```python
from build123d import *

# Parameters (mm, degrees)
SKETCH1_R                  = 50
BOSS_EXTRUDE1_DEPTH        = 20
M56X4_0_TAPPED_HOLE1_D     = 52
M56X4_0_TAPPED_HOLE1_DEPTH = 124
M56X4_0_TAPPED_HOLE1_TIP   = 15.622376095
CIRPATTERN1_COUNT          = 4


with BuildPart() as part:
    # Sketch1 → Boss-Extrude1 (new body)
    with BuildSketch(Plane(origin=(0, 0, 0), x_dir=(1, 0, 0), z_dir=(0, 1, 0))):
        with Locations(Location((0, 0, 0), (0, 0, 270))):
            Circle(SKETCH1_R)
    extrude(amount=BOSS_EXTRUDE1_DEPTH)

    # M56x4.0 Tapped Hole1
    with Locations(Plane(origin=(0, 20, 0), x_dir=(1, 0, 0), z_dir=(0, 1, 0))):
        with Locations((0, 0)):
            Hole(M56X4_0_TAPPED_HOLE1_D / 2, depth=M56X4_0_TAPPED_HOLE1_DEPTH)
            with Locations((0, 0, -(M56X4_0_TAPPED_HOLE1_DEPTH + M56X4_0_TAPPED_HOLE1_TIP / 2))):  # 118° drill point
                Cone(0, M56X4_0_TAPPED_HOLE1_D / 2, M56X4_0_TAPPED_HOLE1_TIP, mode=Mode.SUBTRACT)

    # Sketch5 → Ø14.0 (14) Diameter Hole1 (revolve, cut)
    with BuildSketch(Plane(origin=(0, 10, 50), x_dir=(0, -1, 0), z_dir=(1, 0, 0))):
        Polygon((0, 0), (0, 20), (7, 15.793975667), (7, 0), align=None)
    f_14_0_14_diameter_hole1 = revolve(axis=Axis((0, 10, 56.35), (0, 0, -1)), mode=Mode.SUBTRACT)

    # CirPattern1: Ø14.0 (14) Diameter Hole1 ×4 about axis
    cirpattern1_axis = Axis((0, 20, 0), (0, 1, 0))
    for i in range(1, CIRPATTERN1_COUNT):
        add(f_14_0_14_diameter_hole1.rotate(cirpattern1_axis, i * 360 / CIRPATTERN1_COUNT), mode=Mode.SUBTRACT)


solid = part.part
```
Verification items for the finished model (mm, model axes). A direction names the side the tool comes from. Give positions to 0.01 mm unless a question says otherwise; leave off trailing zeros. Loops run counter-clockwise (first coordinate to the right, second up) from the corner with the lowest first, then second, coordinate; pieces in that order, holes last.
1. Section check C-C, the plane z = 13.5. Enter the section's corners in (x, y), then the cut area to 3 significant figures.
2. Set-up check for faces 5 (the cylindrical face through (-42.214, 3.323, -2.103)), 6 (the conical face through (0.47, 8.88, 30.73)), 7 (the cylindrical face through (42.214, 3.534, -2.681)): record each of +Z, -Z, +X, -X, +Y, -Y from which the full face is reachable in a straight line by a thin tool's end or side.
3. Go/stop test with flat-tipped pins: pin 1 Ø4 at (x, y) = (22.5, 8) entering from -Z; pin 2 Ø11 at (y, z) = (10, 0) entering from +X; pin 3 Ø2 at (x, y) = (-12, 12.5) entering from -Z (3 decimals); pin 4 Ø12 at (x, z) = (-15, 7.5) entering from +Y. Record where each tip stops, or that it passes through.
4. Section check A-A, the plane z = -14.5. Enter the section's corners in (x, y).
5. Thickness scan on line 1 (Y direction, x = -46, z = 0); line 2 (Y direction, x = 39.5, z = 1.5); line 3 (Z direction, x = 38.75, y = 10). Record the ranges inside material, lowest first.
6. Mould release check, pull along Y, two halves, no side actions. Record for faces 1 (the cylindrical face through (2.681, 3.534, 42.214)), 2 (the cylindrical face through (20.633, 9.86, 15.821)), 3 (the flat face through (-22, 0, 22)), 4 (the cylindrical face through (2.103, 3.323, -42.214)): released by +Y, released by -Y, zero draft, split by the parting line, or undercut.
7. Section check B-B, the plane z = 37. Enter the section's corners in (x, y).
Geometry says:
1. outline: (-48.14, 0) - (-22.22, 0) - (-22.22, 20) - (-48.14, 20) - close; (22.22, 0) - (48.14, 0) - (48.14, 20) - (22.22, 20) - close
1. area: 1,040 mm2
2. face 5: -X
2. face 6: +Z
2. face 7: +X
3. pin 1: stops at z = -45.6
3. pin 2: stops at x = 33.3
3. pin 3: stops at z = -48.775
3. pin 4: passes through
4. outline: (-47.85, 0) - (-21.58, 0) - (-21.58, 20) - (-47.85, 20) - close; (21.58, 0) - (47.85, 0) - (47.85, 20) - (21.58, 20) - close
5. line 1: y = 0 to 3, 17 to 20
5. line 2: y = 0 to 3.16, 16.84 to 20
5. line 3: z = -31.6 to -7, 7 to 31.6
6. face 1: undercut
6. face 2: zero draft
6. face 3: released by -Y
6. face 4: undercut
7. outline: (-33.63, 0) - (33.63, 0) - (33.63, 20) - (-33.63, 20) - close; hole circle Ø14 at (0, 10)
